Check sheet for the modelled part. Datum: model origin and axes. Units: mm. Coordinates: 2 decimals unless noted, no trailing zeros. Order: outer loops, then holes, each group sorted by start corner. A loop starts at its lowest first (then second) coordinate and runs counter-clockwise, first axis right, second up. Notation, with made-up numbers: M 45,-20.5 L 50,-20.5 A19 ccw 50,-6.5 Z; hole C 68.25,62.5 d7. An arc over 180 degrees is marked long. Answer in a Markdown table with one row per item. Add a question column.
from build123d import *

# Parameters (mm, degrees)
SKETCH1_W           = 100
SKETCH1_H           = 80
BOSS_EXTRUDE1_DEPTH = 6
SKETCH2_R           = 6.5
CUT_EXTRUDE1_DEPTH  = 6


with BuildPart() as part:
    # Sketch1 → Boss-Extrude1 (new body)
    with BuildSketch(Plane.XY):
        Rectangle(SKETCH1_W, SKETCH1_H)
    extrude(amount=BOSS_EXTRUDE1_DEPTH)

    # Sketch2 → Cut-Extrude1 (cut)
    with BuildSketch(Plane.XY.offset(6)):
        with Locations((-37.5, 27.5)):
            Circle(SKETCH2_R)
        with Locations((37.5, 27.5)):
            Circle(SKETCH2_R)
        with Locations((37.5, -27.5)):
            Circle(SKETCH2_R)
        with Locations((-37.5, -27.5)):
            Circle(SKETCH2_R)
    extrude(amount=-CUT_EXTRUDE1_DEPTH, mode=Mode.SUBTRACT)


solid = part.part
1. Go/stop test with a flat-tipped pin: pin 1 Ø6 at (x, y) = (-14.5, 25.5) entering from -Z. Record where the tip stops, or that it passes through.
2. Section check A-A on x = -37.5. Enter the section's corners in (y, z).
3. Section check B-B on y = 27.5. Enter the section's corners in (x, z).
4. Scan lines: line 1 (Y direction, x = -37, z = 5.15); line 2 (X direction, y = -25, z = 1.45); line 3 (Y direction, x = -43, z = 1.05). Record each from-to range of solid material in increasing order.
5. Section check C-C on z = 4.2. Enter the section's corners in (x, y).
6. Release check for a two-part mould opening along Y. For faces 1 (the flat face through (-50, -1, 3)), 2 (the flat face through (-1, -40, 3)), 3 (the cylindrical face through (31.006, 27.786, 3.042)) record: released by +Y, released by -Y, zero draft, split by the parting line, or undercut.
Result sheet:
| question | item | result |
|---|---|---|
| 1 | pin 1 | z = 0 |
| 2 | outline | M -40,0 L -34,0 L -34,6 L -40,6 Z; M -21,0 L 21,0 L 21,6 L -21,6 Z; M 34,0 L 40,0 L 40,6 L 34,6 Z |
| 3 | outline | M -50,0 L -44,0 L -44,6 L -50,6 Z; M -31,0 L 31,0 L 31,6 L -31,6 Z; M 44,0 L 50,0 L 50,6 L 44,6 Z |
| 4 | line 1 | -40 to -33.98, -21.02 to 21.02, 33.98 to 40 |
| 4 | line 2 | -50 to -43.5, -31.5 to 31.5, 43.5 to 50 |
| 4 | line 3 | -40 to -30.96, -24.04 to 24.04, 30.96 to 40 |
| 5 | outline | M -50,-40 L 50,-40 L 50,40 L -50,40 Z; hole C -37.5,-27.5 d13; hole C -37.5,27.5 d13; hole C 37.5,-27.5 d13; hole C 37.5,27.5 d13 |
| 6 | face 1 | zero draft |
| 6 | face 2 | released by -Y |
| 6 | face 3 | undercut |
